Work out the finished part from the listing and answer in its coordinate system (mm). A direction names the side the tool comes from. Give positions to 0.01 mm unless a question says otherwise; leave off trailing zeros. Loops run counter-clockwise (first coordinate to the right, second up) from the corner with the lowest first, then second, coordinate; pieces in that order, holes last. Notation, with made-up numbers: (51.25, 44.25) - (86.25, 44.25) arc R19 ccw to (86.25, 78.25) - close; hole circle Ø5 at (57.25, 27). An arc over 180 degrees is marked (long way). One line per item, written item: value.
from build123d import *

# Parameters (mm, degrees)
SKETCH1_R            = 6.5
BOSS_EXTRUDE1_DEPTH  = 28
CUT_EXTRUDE1_START   = -14
SKETCH2_W            = 65.403152184
SKETCH2_H            = 73.649752858
CUT_EXTRUDE1_DEPTH   = 28
CUT_EXTRUDE2_DEPTH   = 28
MIRROR2_COPY_1_DEPTH = 28
CHAMFER1_SIZE        = 1
CUT_EXTRUDE3_START   = -14
SKETCH6_W            = 28.147073634
SKETCH6_H            = 26.396452471
CUT_EXTRUDE3_DEPTH   = 28


with BuildPart() as part:
    # Sketch1 → Boss-Extrude1 (new, symmetric)
    with BuildSketch(Plane.XY):
        Polygon((20, 11), (-20, 11), (-39, -8), (-39, -28.882250994), (-33.884776311, -33.997474683), (-18, -18.112698372), (-18, -11), (18, -11), (18, -18.112698372), (33.884776311, -33.997474683), (39, -28.882250994), (39, -8), align=None)
        Circle(SKETCH1_R, mode=Mode.SUBTRACT)
    extrude(amount=BOSS_EXTRUDE1_DEPTH, both=True)

    # Sketch2 → Cut-Extrude1 (cut)
    with BuildSketch(Plane.XY.offset(28).offset(CUT_EXTRUDE1_START)):
        with Locations((-20.201576092, 0)):
            Rectangle(SKETCH2_W, SKETCH2_H)
    extrude(amount=-CUT_EXTRUDE1_DEPTH, mode=Mode.SUBTRACT)

    # Sketch5 → Cut-Extrude2 (cut)
    with BuildSketch(Plane(origin=(-33.941125497, -33.941125497, 0), x_dir=(0, 0, 1), z_dir=(-0.7071067811865506, -0.7071067811865445, 0))):
        Polygon((-22.833333333, -0.079689783), (-19.166666667, -0.079689783), (-21, 1.216672649), align=None)
        Polygon((-17.666666667, -0.079689783), (-14, -0.079689783), (-15.833333333, 1.216672649), align=None)
        Polygon((-24.333333333, -0.079689783), (-26.166666667, 1.216672649), (-28, -0.079689783), align=None)
    cut_extrude2 = extrude(amount=-CUT_EXTRUDE2_DEPTH, mode=Mode.SUBTRACT)

    # Mirror1: Cut-Extrude2 across plane
    add(cut_extrude2.mirror(Plane.XY), mode=Mode.SUBTRACT)

    # Mirror2: Cut-Extrude2 across plane
    add(cut_extrude2.mirror(Plane(origin=(0, 0, 0), x_dir=(0, 0, 1), z_dir=(1, 0, 0))), mode=Mode.SUBTRACT)

    # Mirror2 copy 1 sketch → Mirror2 copy 1 (cut)
    with BuildSketch(Plane(origin=(33.941125497, -33.941125497, 0), x_dir=(0, 0, -1), z_dir=(0.7071067811865506, -0.7071067811865445, 0))):
        Polygon((-22.833333333, -0.079689783), (-19.166666667, -0.079689783), (-21, 1.216672649), align=None)
        Polygon((-17.666666667, -0.079689783), (-14, -0.079689783), (-15.833333333, 1.216672649), align=None)
        Polygon((-24.333333333, -0.079689783), (-26.166666667, 1.216672649), (-28, -0.079689783), align=None)
    extrude(amount=-MIRROR2_COPY_1_DEPTH, mode=Mode.SUBTRACT)

    # Chamfer1
    chamfer1_edges = [part.edges().sort_by_distance(p)[0] for p in [
        (-6.5, 0, -28),
        (-6.5, 0, 28),
    ]]
    chamfer(chamfer1_edges, length=CHAMFER1_SIZE)

    # Sketch6 → Cut-Extrude3 (cut)
    with BuildSketch(Plane.XY.offset(28).offset(CUT_EXTRUDE3_START)):
        with Locations((32.073536817, -24.198226236)):
            Rectangle(SKETCH6_W, SKETCH6_H)
    extrude(amount=-CUT_EXTRUDE3_DEPTH, mode=Mode.SUBTRACT)


solid = part.part
1. Section B-B (x = 0) is taken. Write down the section's boundary in (y, z), and give its area (3 significant figures).
Output:
outline: (-11, -28) - (-7.5, -28) - (-6.5, -27) - (-6.5, -14) - (-11, -14) - close; (-11, 14) - (-6.5, 14) - (-6.5, 27) - (-7.5, 28) - (-11, 28) - close; (6.5, -27) - (7.5, -28) - (11, -28) - (11, -14) - (6.5, -14) - close; (6.5, 14) - (11, 14) - (11, 28) - (7.5, 28) - (6.5, 27) - close
area: 250 mm²
2. Section C-C (y = -12) is taken. Write down the section's boundary in (x, z).
Output:
outline: (-39, -28) - (-18, -28) - (-18, -14) - (-39, -14) - close; (-39, 14) - (-18, 14) - (-18, 28) - (-39, 28) - close; (18, -28) - (39, -28) - (39, -14) - (18, -14) - close; (18, 14) - (39, 14) - (39, 28) - (18, 28) - close
3. Section A-A (y = 0) is taken. Write down the section's boundary in (x, z), and give its area (3 significant figures).
Output:
outline: (-31, -28) - (-7.5, -28) - (-6.5, -27) - (-6.5, -14) - (-31, -14) - close; (-31, 14) - (-6.5, 14) - (-6.5, 27) - (-7.5, 28) - (-31, 28) - close; (6.5, -27) - (7.5, -28) - (31, -28) - (31, 28) - (7.5, 28) - (6.5, 27) - (6.5, 14) - (12.5, 14) - (12.5, -14) - (6.5, -14) - close
area: 1,890 mm²
4. Find the intervals of material crossed by line 1 along X through (y, z) = (-12.5, -20); line 2 along Z through (x, y) = (-21.5, -6.5); line 3 along Y through (x, z) = (0, 17.25), in increasing order.
Output:
line 1: x = -39 to -18, 18 to 39
line 2: z = -28 to -14, 14 to 28
line 3: y = -11 to -6.5, 6.5 to 11
5. The mould has two halves that part along X. Classify faces 4 (the flat face through (-29, 2, 21)), 5 (the flat face through (-26.054, -26.166, -23.573)), 6 (the flat face through (31, -20, -14)): released by +X, released by -X, zero draft, split by the parting line, or undercut.
Output:
face 4: released by -X
face 5: undercut
face 6: zero draft
6. Section D-D (z = -13) is taken. Write down the section's boundary in (x, y).
Output:
outline: (12.5, -11) - (39, -11) - (39, -8) - (20, 11) - (12.5, 11) - close
7. Flat-ended cylindrical pins translate along their axes: pin 1 Ø11 at (y, z) = (1, 2) entering from -X; pin 2 Ø2 at (x, z) = (23.5, -11) entering from +Y; pin 3 Ø5 at (y, z) = (6.5, 2) entering from +X; pin 4 Ø6 at (y, z) = (-18.5, 9.5) entering from -X. Find the tip coordinate at first contact, or state that the pin passes through.
Output:
pin 1: stops at x = 12.5
pin 2: stops at y = 8.5
pin 3: stops at x = 27
pin 4: passes through
8. For faces 1 (the flat face through (-26.054, -26.166, 18.427)), 2 (the flat face through (-26.05, -25.26, 20.07)), 3 (the flat face through (36.407, -31.476, 21.098)), determine the directions among +Z, -Z, +X, -X, +Y, -Y from which every point of the face is accessible in a straight line to the end or side of a thin tool.
Output:
face 1: +Z, -Z, -Y
face 2: -Y
face 3: +Z, -Z, +X, -Y
